Geometry: final body of the model. Coordinates: model frame, mm. Face numbers are marked on the shaded views. Give positions to 0.01 mm unless a question says otherwise; leave off trailing zeros. Write each loop counter-clockwise with the first axis right and the second up, starting at its lowest first coordinate (ties: lowest second). Pieces come first, ordered by that corner, then holes. Notation, with made-up numbers: (12, 79.25) -> (52, 79.25) arc R18 cw to (52, 114.25) -> close; hole circle Ø10 at (67, 17). An arc over 180 degrees is marked (long way). Answer in a Markdown table with one row per item. Add a question column.
Item 1: Section query D-D on z = 5.5. Output: boundary loops of the cut face in (x, y), plus the area to 3 significant figures.
Item 2: Section query B-B on x = 0. Output: boundary loops of the cut face in (y, z).
Item 3: Section query C-C on z = 18. Output: boundary loops of the cut face in (x, y), plus the area to 3 significant figures.
Item 4: Section query A-A on y = 0. Output: boundary loops of the cut face in (x, z), plus the area to 3 significant figures.
Item 5: Material intervals for probe 1 along Z at (x, y) = (0, 38); probe 2 along Y at (x, z) = (0, 8); probe 3 along X at (y, z) = (-1, 21), sorted ascending. Write a range as from..to.
Item 6: Draft query along X for the marked faces 1, 2 and 3. Return one class per face: +X half, -X half, draft (parallel to the pull), parting line (faces both ways), or undercut.
Item 7: First-contact query: P1, Ø1, axis at y = -15.5, z = 7, coming from the -X side; P2, Ø2, axis at y = -13, z = 16.5, coming from the -X side; P3, Ø4, axis at y = -24.5, z = 21.5, coming from the +X side; P4, Ø12, axis at x = 29, y = -6.5, coming from the -Z side. Flat tips, straight axial feed; report the tip coordinate or a pass-through.
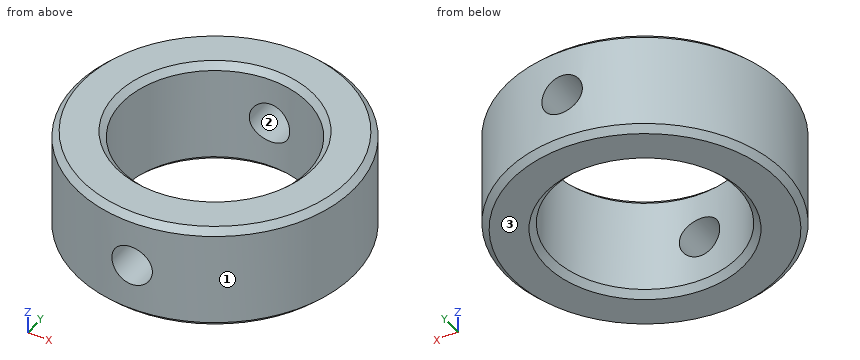
```python
from build123d import *

# Parameters (mm, degrees)
SKETCH1_R               = 45
SKETCH1_R_2             = 30
BOSS_EXTRUDE1_DEPTH     = 34
CUT_EXTRUDE1_DEPTH      = 73.15261603
CUT_EXTRUDE1_DEPTH_BACK = 73.15261603
SKETCH2_R               = 6.5
CHAMFER1_SIZE           = 2


with BuildPart() as part:
    # Sketch1 → Boss-Extrude1 (new body)
    with BuildSketch(Plane.XY):
        Circle(SKETCH1_R)
        Circle(SKETCH1_R_2, mode=Mode.SUBTRACT)
    extrude(amount=BOSS_EXTRUDE1_DEPTH)

    # Sketch2 → Cut-Extrude1 (cut, two sides: drawn at the far end of the back side and taken through both)
    with BuildSketch(Plane(origin=(0, 0, 0), x_dir=(1, 0, 0), z_dir=(0, 1, 0)).offset(-CUT_EXTRUDE1_DEPTH_BACK)):
        with Locations(Location((0, -17, 0), (0, 0, 270))):
            Circle(SKETCH2_R)
    extrude(amount=CUT_EXTRUDE1_DEPTH + CUT_EXTRUDE1_DEPTH_BACK, mode=Mode.SUBTRACT)

    # Chamfer1
    chamfer1_edges = [part.edges().sort_by_distance(p)[0] for p in [
        (-45, 0, 0),
        (-45, 0, 34),
        (-30, 0, 0),
        (-30, 0, 34),
    ]]
    chamfer(chamfer1_edges, length=CHAMFER1_SIZE)


solid = part.part
```
Findings below:
| question | item | result |
|---|---|---|
| 1 | outline | circle Ø90 at (0, 0); hole circle Ø60 at (0, 0) |
| 1 | area | 3,530 mm^2 |
| 2 | outline | (-45, 2) -> (-43, 0) -> (-32, 0) -> (-30, 2) -> (-30, 10.5) -> (-45, 10.5) -> close; (-45, 23.5) -> (-30, 23.5) -> (-30, 32) -> (-32, 34) -> (-43, 34) -> (-45, 32) -> close; (30, 2) -> (32, 0) -> (43, 0) -> (45, 2) -> (45, 10.5) -> (30, 10.5) -> close; (30, 23.5) -> (45, 23.5) -> (45, 32) -> (43, 34) -> (32, 34) -> (30, 32) -> close |
| 3 | outline | (-6.42, -44.54) -> (-6.42, -29.3) arc R30 cw to (-6.42, 29.3) -> (-6.42, 44.54) arc R45 ccw to start; (6.42, -44.54) arc R45 ccw to (6.42, 44.54) -> (6.42, 29.3) arc R30 cw to (6.42, -29.3) -> close |
| 3 | area | 3,150 mm^2 |
| 4 | outline | (-45, 2) -> (-43, 0) -> (-32, 0) -> (-30, 2) -> (-30, 32) -> (-32, 34) -> (-43, 34) -> (-45, 32) -> close; (30, 2) -> (32, 0) -> (43, 0) -> (45, 2) -> (45, 32) -> (43, 34) -> (32, 34) -> (30, 32) -> close |
| 4 | area | 1,000 mm^2 |
| 5 | probe 1 | z = 0..10.5, 23.5..34 |
| 5 | probe 2 | y = -45..-30, 30..45 |
| 5 | probe 3 | x = -44.99..-29.98, 29.98..44.99 |
| 6 | face 1 | parting line |
| 6 | face 2 | undercut |
| 6 | face 3 | draft |
| 7 | P1 | stops at x = -42.43 |
| 7 | P2 | stops at x = -43.37 |
| 7 | P3 | stops at x = 38.97 |
| 7 | P4 | stops at z = 0 |
